```python
from build123d import *

# Parameters (mm, degrees)
EXTRUDE_1_DEPTH     = 10
SKETCH_2_R          = 2
CUT_EXTRUDE_1_DEPTH = 34
SKETCH_3_W          = 16
SKETCH_3_H          = 87.857567692
CUT_EXTRUDE_2_DEPTH = 17
SKETCH_5_W          = 20
SKETCH_5_H          = 20
EXTRUDE_2_DEPTH     = 2
SKETCH_6_R          = 5
EXTRUDE_3_DEPTH     = 200
SKETCH_7_R          = 2
CUT_EXTRUDE_3_DEPTH = 30.5


with BuildPart() as part:
    # Sketch 1 → Extrude 1 (new, symmetric)
    with BuildSketch(Plane.XY):
        with BuildLine():
            Line((-10, 20), (-10, 0))
            Line((-10, 0), (10, 0))
            Line((10, 0), (10, 20))
            ThreePointArc((10, 20), (0, 30), (-10, 20))
        make_face()
    extrude(amount=EXTRUDE_1_DEPTH, both=True)

    # Sketch 2 → Cut-Extrude 1 (cut)
    with BuildSketch(Plane(origin=(0, 0, -10), x_dir=(-1, 0, 0), z_dir=(0, 0, -1))):
        with Locations((0, 20)):
            Circle(SKETCH_2_R)
    extrude(amount=-CUT_EXTRUDE_1_DEPTH, mode=Mode.SUBTRACT)

    # Sketch 3 → Cut-Extrude 2 (cut, symmetric)
    with BuildSketch(Plane(origin=(0, 0, 0), x_dir=(0, 0, -1), z_dir=(1, 0, 0))):
        Rectangle(SKETCH_3_W, SKETCH_3_H)
    extrude(amount=CUT_EXTRUDE_2_DEPTH, both=True, mode=Mode.SUBTRACT)


with BuildPart() as cut_extrude_2_piece_1:
    # of the separate pieces the step leaves, piece 1, a body of its own (cut_extrude_2_pieces)
    add(part.part.solids().sort_by_distance((-10, 20, -8))[0])



with BuildPart() as cut_extrude_2_piece_2:
    # of the separate pieces the step leaves, piece 2, a body of its own (cut_extrude_2_pieces)
    add(part.part.solids().sort_by_distance((-10, 20, 10))[0])


with BuildPart() as cut_extrude_2_piece_1_1:
    add(cut_extrude_2_piece_1.part)

    add(cut_extrude_2_piece_2.part)  # Extrude 2 merges Cut-Extrude 2 piece 2
    # Sketch 5 → Extrude 2 (add)
    with BuildSketch(Plane.XZ):
        Rectangle(SKETCH_5_W, SKETCH_5_H)
    extrude(amount=EXTRUDE_2_DEPTH)

    # Sketch 6 → Extrude 3 (add)
    with BuildSketch(Plane.XZ.offset(2)):
        with Locations(Location((0, 0, 0), (0, 0, 270))):
            Circle(SKETCH_6_R)
    extrude(amount=EXTRUDE_3_DEPTH)

    # Sketch 7 → Cut-Extrude 3 (cut, symmetric)
    with BuildSketch(Plane.XY):
        with Locations(Location((0, -193.17530314, 0), (0, 0, 269.999999999))):
            Circle(SKETCH_7_R)
    extrude(amount=CUT_EXTRUDE_3_DEPTH, both=True, mode=Mode.SUBTRACT)


solid = cut_extrude_2_piece_1_1.part
```
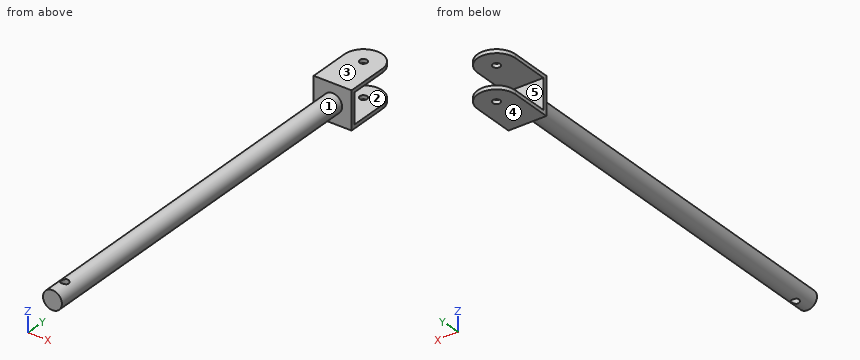
Here's how the part is built. I have some questions about the finished solid (model axes, mm). Face numbers are marked on the shaded views. A direction names the side the tool comes from. Give positions to 0.01 mm unless a question says otherwise; leave off trailing zeros. Order: outer loops, then holes, each group sorted by start corner. A loop starts at its lowest first (then second) coordinate and runs counter-clockwise, first axis right, second up. Notation, with made-up numbers: (-5.75, 35.25) - (43.25, 35.25) arc R11 ccw to (43.25, 53.25) - close; hole circle Ø5 at (82, -3). An arc over 180 degrees is marked (long way). Answer as a JSON object with one key per item and string values. Group by question number.
Item 1: Which directions (+Z, -Z, +X, -X, +Y, -Y) give clear straight access to the entire face, cutting with the end or side of a thin tool? Please do the marked faces 4 and 5.
Item 2: If we mould it in two halves opening along Z, with no side actions, what happens to the marked faces 1, 2 and 3? For each: pulls with the +Z half, pulls with the -Z half, needs draft (parallel to the pull), parting line crosses it, or undercut.
Item 3: If we section it at A-A on x = 0: Please give me the cut outline in (y, z).
Item 4: For P1, Ø3, axis at x = -3, z = -6, coming from the -Y side; P2, Ø1.5, axis at x = 5, z = 7, coming from the +Y side; P3, Ø10, axis at x = -3.5, y = -63.5, coming from the -Z side; P4, Ø2, axis at y = -166, z = 7, coming from the -X side, each with a flat end and sliding along its axis, tell me the tip position at first contact or that it passes through.
Item 5: Please list where these lines run through material, in increasing order: probe 1 along Y at (x, z) = (0, -2.25); probe 2 along Z at (x, y) = (8, 8); probe 3 along Y at (x, z) = (0, -8.35).
Item 6: If we section it at C-C on y = -77: Please give me the cut outline in (x, z).
Item 7: If we section it at B-B on z = -0.75: Please give me the cut outline in (x, y), and give its area (3 significant figures).
Result set:
{
 "1": {"face 4": "-Z, +X, -X, +Y, -Y", "face 5": "+X, -X, +Y"},
 "2": {"face 1": "parting line crosses it", "face 2": "undercut", "face 3": "pulls with the +Z half"},
 "3": {"outline": "(-202, -5) - (-195.18, -5) - (-195.18, 5) - (-202, 5) - close; (-191.18, -5) - (-2, -5) - (-2, -10) - (18, -10) - (18, -8) - (0, -8) - (0, 8) - (18, 8) - (18, 10) - (-2, 10) - (-2, 5) - (-191.18, 5) - close; (22, -10) - (30, -10) - (30, -8) - (22, -8) - close; (22, 8) - (30, 8) - (30, 10) - (22, 10) - close"},
 "4": {"P1": "y = -2", "P2": "y = 0", "P3": "z = -5", "P4": "through"},
 "5": {"probe 1": "-202 to -195.18, -191.18 to 0", "probe 2": "-10 to -8, 8 to 10", "probe 3": "-2 to 18, 22 to 30"},
 "6": {"outline": "circle Ø10 at (0, 0)"},
 "7": {"outline": "(-10, -2) - (-4.94, -2) - (-4.94, -202) - (4.94, -202) - (4.94, -2) - (10, -2) - (10, 0) - (-10, 0) - close; hole circle Ø4 at (0, -193.18)", "area": "2,000 mm²"}
}
